```python
from build123d import *

# Parameters (mm, degrees)
BASE_PLATE_6MM_DEPTH      = 6
GUIDE_UPRIGHTS_17MM_DEPTH = 17
UPRIGHT_FILLETS_R5_R      = 5
UPRIGHT_CUT_A_DEPTH       = 17
UPRIGHT_CUT_B_DEPTH       = 17
UPRIGHT_CUT_C_DEPTH       = 17


with BuildPart() as part:
    # Bracket Profile Sketch → Base Plate 6mm (new body)
    with BuildSketch(Plane(origin=(0, 0, 0), x_dir=(1, 0, 0), z_dir=(0, 1, 0))):
        with BuildLine():
            Line((10, 6), (10, 0))
            Line((10, 0), (30, 0))
            Line((30, 0), (30, 6))
            Line((30, 6), (38.5, 6))
            ThreePointArc((38.5, 6), (34.964466094, 7.464466094), (33.5, 11))
            Line((33.5, 11), (33.5, 12))
            ThreePointArc((33.5, 12), (31.742640687, 16.242640687), (27.5, 18))
            Line((27.5, 18), (12.5, 18))
            ThreePointArc((12.5, 18), (8.257359313, 16.242640687), (6.5, 12))
            Line((6.5, 12), (6.5, 11))
            ThreePointArc((6.5, 11), (5.035533906, 7.464466094), (1.5, 6))
            Line((1.5, 6), (10, 6))
        make_face()
        with BuildLine():
            ThreePointArc((12.5, 9), (9.5, 12), (12.5, 15))
            Line((12.5, 15), (27.5, 15))
            ThreePointArc((27.5, 15), (30.5, 12), (27.5, 9))
            Line((27.5, 9), (12.5, 9))
        make_face(mode=Mode.SUBTRACT)
    extrude(amount=BASE_PLATE_6MM_DEPTH)

    # Sketch1_3 → Guide Uprights 17mm (add)
    with BuildSketch(Plane(origin=(0, 0, 0), x_dir=(1, 0, 0), z_dir=(0, 1, 0))):
        Polygon((30, 6), (30, 0), (40, 0), (40, 6), (38.5, 6), align=None)
        Polygon((0, 6), (0, 0), (10, 0), (10, 6), (1.5, 6), align=None)
    extrude(amount=GUIDE_UPRIGHTS_17MM_DEPTH)

    # Upright Fillets R5
    upright_fillets_r5_edges = [part.edges().sort_by_distance(p)[0] for p in [
        (10, 6, -3),
        (30, 6, -3),
    ]]
    fillet(upright_fillets_r5_edges, radius=UPRIGHT_FILLETS_R5_R)

    # Upright Cut Profiles Sketch → Upright Cut A (cut)
    with BuildSketch(Plane(origin=(0, 0, -6), x_dir=(-1, 0, 0), z_dir=(0, 0, -1))):
        with BuildLine():
            Line((-32.5, 11.844225053), (-35, 11.844225053))
            Line((-35, 11.844225053), (-37.497250612, 11.961440165))
            ThreePointArc((-37.497250612, 11.961440165), (-35.058623676, 9.344912495), (-32.5, 11.844225053))
        make_face()
        with BuildLine():
            Line((-37.497250612, 11.961440165), (-35, 11.844225053))
            Line((-35, 11.844225053), (-32.5, 11.844225053))
            ThreePointArc((-32.5, 11.844225053), (-34.941376324, 14.343537612), (-37.497250612, 11.961440165))
        make_face()
        with BuildLine():
            Line((-32.5, 11.844225053), (-35, 11.844225053))
            Line((-35, 11.844225053), (-37.497250612, 11.961440165))
            ThreePointArc((-37.497250612, 11.961440165), (-35.058623676, 9.344912495), (-32.5, 11.844225053))
        make_face()
        with BuildLine():
            Line((-37.497250612, 11.961440165), (-35, 11.844225053))
            Line((-35, 11.844225053), (-32.5, 11.844225053))
            ThreePointArc((-32.5, 11.844225053), (-34.941376324, 14.343537612), (-37.497250612, 11.961440165))
        make_face()
        with BuildLine():
            Line((-2.5, 11.844225053), (-5, 11.844225053))
            Line((-5, 11.844225053), (-7.5, 11.844225053))
            ThreePointArc((-7.5, 11.844225053), (-5, 9.344225053), (-2.5, 11.844225053))
        make_face()
        with BuildLine():
            Line((-7.5, 11.844225053), (-5, 11.844225053))
            Line((-5, 11.844225053), (-2.5, 11.844225053))
            ThreePointArc((-2.5, 11.844225053), (-5, 14.344225053), (-7.5, 11.844225053))
        make_face()
        with BuildLine():
            Line((-2.5, 11.844225053), (-5, 11.844225053))
            Line((-5, 11.844225053), (-7.5, 11.844225053))
            ThreePointArc((-7.5, 11.844225053), (-5, 9.344225053), (-2.5, 11.844225053))
        make_face()
        with BuildLine():
            Line((-7.5, 11.844225053), (-5, 11.844225053))
            Line((-5, 11.844225053), (-2.5, 11.844225053))
            ThreePointArc((-2.5, 11.844225053), (-5, 14.344225053), (-7.5, 11.844225053))
        make_face()
    extrude(amount=-UPRIGHT_CUT_A_DEPTH, mode=Mode.SUBTRACT)

    # Sketch2_7 → Upright Cut B (cut)
    with BuildSketch(Plane(origin=(0, 0, -6), x_dir=(-1, 0, 0), z_dir=(0, 0, -1))):
        with BuildLine():
            ThreePointArc((0, 11.844225053), (-5, 16.844225053), (-10, 11.844225053))
            Line((-10, 11.844225053), (-10, 17))
            Line((-10, 17), (0, 17))
            Line((0, 17), (0, 11.844225053))
        make_face()
    extrude(amount=-UPRIGHT_CUT_B_DEPTH, mode=Mode.SUBTRACT)

    # Sketch2_12 → Upright Cut C (cut)
    with BuildSketch(Plane(origin=(0, 0, -6), x_dir=(-1, 0, 0), z_dir=(0, 0, -1))):
        with BuildLine():
            Line((-40, 17), (-39.994501223, 12.078655276))
            ThreePointArc((-39.994501223, 12.078655276), (-34.882752648, 16.84285017), (-30, 11.844225053))
            Line((-30, 11.844225053), (-30, 17))
            Line((-30, 17), (-40, 17))
        make_face()
    extrude(amount=-UPRIGHT_CUT_C_DEPTH, mode=Mode.SUBTRACT)


solid = part.part
```
Build history of the part. All positions in model axes, mm. A direction names the side the tool comes from. Coordinates: 2 decimals unless noted, no trailing zeros. Write each loop counter-clockwise with the first axis right and the second up, starting at its lowest first coordinate (ties: lowest second). Pieces come first, ordered by that corner, then holes.
1. Band-saw the part on B-B, the plane x = 22. Give the cut face in (y, z).
Answer block:
outline: (0, -18) - (6, -18) - (6, -15) - (0, -15) - close; (0, -9) - (6, -9) - (6, 0) - (0, 0) - close
2. Pull direction X, two halves, no side cores. Call faces 1 (the cylindrical face through (2.615, 12.595, -3.042)), 2 (the flat face through (6, 8, -6)), 3 (the cylindrical face through (31.789, 2.958, -16.196)): released by +X, released by -X, zero draft, split by the parting line, or undercut.
Answer block:
face 1: undercut
face 2: zero draft
face 3: released by +X
3. Band-saw the part on D-D, the plane y = 9.75. Give the cut face in (x, z), and give its area (3 significant figures).
Answer block:
outline: (0, -6) - (3.63, -6) - (3.63, 0) - (0, 0) - close; (6.37, -6) - (10.16, -6) - (10.16, 0) - (6.37, 0) - close; (29.84, -6) - (33.63, -6) - (33.63, 0) - (29.84, 0) - close; (36.37, -6) - (40, -6) - (40, 0) - (36.37, 0) - close
area: 89.1 mm2
4. Band-saw the part on C-C, the plane y = 1.5. Give the cut face in (x, z).
Answer block:
outline: (0, -6) - (1.5, -6) arc R5 cw to (6.5, -11) - (6.5, -12) arc R6 ccw to (12.5, -18) - (27.5, -18) arc R6 ccw to (33.5, -12) - (33.5, -11) arc R5 cw to (38.5, -6) - (40, -6) - (40, 0) - (0, 0) - close; hole (12.5, -15) - (27.5, -15) arc R3 ccw to (27.5, -9) - (12.5, -9) arc R3 ccw to start
5. 3-axis set-ups, long thin cutter, end or side, ignore diameter. For faces 4 (the flat face through (20, 5, 0)), 5 (the flat face through (20, 6, -7)), 6 (the cylindrical face through (29, 8, -3)), 7 (the flat face through (20, 3, -9)), 8 (the flat face through (20, 0, -7)): which of +Z, -Z, +X, -X, +Y, -Y reach the whole face in a straight line?
Answer block:
face 4: +Z, +X, -X, +Y, -Y
face 5: -Z, +Y
face 6: +Z, -Z, +Y
face 7: +Y, -Y
face 8: +Z, -Z, +X, -X, -Y
6. Drop flat-ended pins along their axis: pin 1 (10 mm diameter, centred on x = 20, z = -2.5, fed in from +Y); pin 2 (4.5 mm diameter, centred on x = 34.5, y = 11.5, fed in from -Z); pin 3 (2 mm diameter, centred on x = 35, z = -13.5, fed in from -Y); pin 4 (0.5 mm diameter, centred on y = 4, z = -11.5, fed in from -X). Give the stop position or say it passes through.
Answer block:
pin 1: stops at y = 6
pin 2: stops at z = -6
pin 3: passes through
pin 4: stops at x = 6.5
7. Drill centre lines: probe 1 along Y at (x, z) = (5, -2.2); probe 2 along X at (y, z) = (11.75, -3.75); probe 3 along Z at (x, y) = (19, 5.75). Where is each one in solid material? Low to high.
Answer block:
probe 1: y = 0 to 9.34, 14.34 to 16.84
probe 2: x = 0 to 2.5, 7.5 to 10, 30 to 32.5, 37.5 to 40
probe 3: z = -18 to -15, -9 to 0
8. Band-saw the part on A-A, the plane z = -2.5. Give the cut face in (x, y), and give its area (3 significant figures).
Answer block:
outline: (0, 0) - (40, 0) - (40, 17) - (39.99, 12.08) arc R5 ccw to (30, 11.84) - (30, 11) arc R5 cw to (25, 6) - (15, 6) arc R5 cw to (10, 11) - (10, 11.84) arc R5 ccw to (0, 11.84) - close; hole circle Ø5 at (5, 11.84); hole circle Ø5 at (35, 11.84)
area: 407 mm2
